Check sheet for the modelled part. Datum: model origin and axes. Units: mm. A direction names the side the tool comes from. Coordinates: 2 decimals unless noted, no trailing zeros. Write each loop counter-clockwise with the first axis right and the second up, starting at its lowest first coordinate (ties: lowest second). Pieces come first, ordered by that corner, then holes. Notation, with made-up numbers: (0.25, -14.5) -> (58.25, -14.5) arc R13 cw to (58.25, 8.5) -> close; hole circle Ø9 at (76.25, 53). An arc over 180 degrees is marked (long way). Put each result on its own line as item: value.
```python
from build123d import *

# Parameters (mm, degrees)
BOSS_EXTRUDE1_DEPTH                                  = 50
CUT_EXTRUDE1_DEPTH                                   = 30
SKETCH3_R                                            = 25
CUT_EXTRUDE2_DEPTH                                   = 30
CBORE_FOR_M6_HEXAGON_HEAD_BOLTS_FULL_THR_D           = 6.6
CBORE_FOR_M6_HEXAGON_HEAD_BOLTS_FULL_THR_CBORE_D     = 13
CBORE_FOR_M6_HEXAGON_HEAD_BOLTS_FULL_THR_CBORE_DEPTH = 0.5
CUT_EXTRUDE8_DEPTH                                   = 30


with BuildPart() as part:
    # Sketch1 → Boss-Extrude1 (new body)
    with BuildSketch(Plane(origin=(0, 0, 0), x_dir=(1, 0, 0), z_dir=(0, 1, 0))):
        with BuildLine():
            Line((-220, -250), (220, -250))
            ThreePointArc((220, -250), (241.213203436, -241.213203436), (250, -220))
            Line((250, -220), (250, 220))
            ThreePointArc((250, 220), (241.213203436, 241.213203436), (220, 250))
            Line((220, 250), (-220, 250))
            ThreePointArc((-220, 250), (-241.213203436, 241.213203436), (-250, 220))
            Line((-250, 220), (-250, -220))
            ThreePointArc((-250, -220), (-241.213203436, -241.213203436), (-220, -250))
        make_face()
    extrude(amount=BOSS_EXTRUDE1_DEPTH)

    # Sketch2 → Cut-Extrude1 (cut)
    with BuildSketch(Plane(origin=(0, 50, 0), x_dir=(1, 0, 0), z_dir=(0, 1, 0))):
        with BuildLine():
            Line((-175, -210), (175, -210))
            ThreePointArc((175, -210), (185.251262658, -185.251262658), (210, -175))
            Line((210, -175), (210, 175))
            ThreePointArc((210, 175), (185.251262658, 185.251262658), (175, 210))
            Line((175, 210), (-175, 210))
            ThreePointArc((-175, 210), (-185.251262658, 185.251262658), (-210, 175))
            Line((-210, 175), (-210, -175))
            ThreePointArc((-210, -175), (-185.251262658, -185.251262658), (-175, -210))
        make_face()
    extrude(amount=-CUT_EXTRUDE1_DEPTH, mode=Mode.SUBTRACT)

    # Sketch3 → Cut-Extrude2 (cut)
    with BuildSketch(Plane.XZ):
        with Locations(Location((-210, 210, 0), (0, 0, 270))):
            Circle(SKETCH3_R)
        with Locations(Location((210, 210, 0), (0, 0, 90))):
            Circle(SKETCH3_R)
        with Locations(Location((210, -210, 0), (0, 0, 270))):
            Circle(SKETCH3_R)
        with Locations(Location((-210, -210, 0), (0, 0, 90))):
            Circle(SKETCH3_R)
    extrude(amount=-CUT_EXTRUDE2_DEPTH, mode=Mode.SUBTRACT)

    # CBORE for M6 Hexagon head bolts-Full thread-grade C1 (through all)
    with Locations(Plane.XZ):
        with Locations((90, 200), (-90, 200), (90, 120), (-90, 120)):
            CounterBoreHole(CBORE_FOR_M6_HEXAGON_HEAD_BOLTS_FULL_THR_D / 2, CBORE_FOR_M6_HEXAGON_HEAD_BOLTS_FULL_THR_CBORE_D / 2, CBORE_FOR_M6_HEXAGON_HEAD_BOLTS_FULL_THR_CBORE_DEPTH)

    # Sketch10 → Cut-Extrude8 (cut)
    with BuildSketch(Plane(origin=(0, 50, 0), x_dir=(1, 0, 0), z_dir=(0, 1, 0))):
        with BuildLine():
            Line((-210, -175), (-210, -210))
            Line((-210, -210), (-175, -210))
            ThreePointArc((-175, -210), (-185.251262658, -185.251262658), (-210, -175))
        make_face()
    extrude(amount=-CUT_EXTRUDE8_DEPTH, mode=Mode.SUBTRACT)


solid = part.part
```
Q1. Cross-section at D-D (x = 24). Record the cut outline in (y, z), plus the area to 3 significant figures.
Recorded:
outline: (0, -250) -> (50, -250) -> (50, -210) -> (20, -210) -> (20, 210) -> (50, 210) -> (50, 250) -> (0, 250) -> close
area: 12,400 mm2
Q2. Cross-section at A-A (z = -37.5). Record the cut outline in (x, y).
Recorded:
outline: (-250, 0) -> (250, 0) -> (250, 50) -> (210, 50) -> (210, 20) -> (-210, 20) -> (-210, 50) -> (-250, 50) -> close
Q3. Mould release check, pull along Z, two halves, no side actions. Record for faces 4 (the flat face through (-3, 25, 250)), 5 (the cylindrical face through (-87.001, 0.246, 194.233)), 6 (the flat face through (3, 25, -250)): released by +Z, released by -Z, zero draft, split by the parting line, or undercut.
Recorded:
face 4: released by +Z
face 5: undercut
face 6: released by -Z
Q4. Material ranges on line 1 along Z through (x, y) = (89.5, 19); line 2 along Z through (x, y) = (-208, 12); line 3 along X through (y, z) = (18, -210), recorded low to high.
Recorded:
line 1: z = -250 to 116.74, 123.26 to 196.74, 203.26 to 250
line 2: z = -250 to -234.92, -185.08 to 185.08, 234.92 to 250
line 3: x = -250 to -235, -185 to 185, 235 to 250
Q5. Depth check by flat-ended pin: P1, Ø6, axis at x = -90, z = 200, coming from the +Y side; P2, Ø6.5, axis at x = -91, z = 203, coming from the -Y side; P3, Ø25, axis at x = -221, z = -205.5, coming from the -Y side; P4, Ø6, axis at x = 7, z = -149, coming from the +Y side. Enter the tip coordinate at first touch or a pass-through.
Recorded:
P1: passes through
P2: stops at y = 0.5
P3: stops at y = 30
P4: stops at y = 20
Q6. Cross-section at C-C (x = -193). Record the cut outline in (y, z), plus the area to 3 significant figures.
Recorded:
outline: (0, -250) -> (50, -250) -> (50, -179.41) -> (20, -179.41) -> (20, 191.67) -> (0, 191.67) -> (0, -191.67) -> (30, -191.67) -> (30, -228.33) -> (0, -228.33) -> close; (0, 228.33) -> (30, 228.33) -> (30, 210) -> (50, 210) -> (50, 250) -> (0, 250) -> close
area: 11,300 mm2
Q7. Tool access check on faces 1 (the flat face through (-3, 20, -3)), 2 (the flat face through (-226, 50, -3)), 3 (the cylindrical face through (-83.8, 0.25, 121.95)). Record the directions out of +Z, -Z, +X, -X, +Y, -Y that give a thin tool (end or side, any length) a straight path to the whole face; none if there is none.
Recorded:
face 1: +Y
face 2: +Z, -Z, +X, -X, +Y
face 3: -Y
Q8. Cross-section at B-B (y = 7.5). State how many separate pieces and enclosed holes the cut face has, plus the area to 3 significant figures.
Recorded:
separate pieces: 1
enclosed holes: 8
area: 241,000 mm2
